For this review, take the finished solid that the model builds, in its own axes (mm). Face numbers are marked on the shaded views. A direction names the side the tool comes from. Coordinates: 2 decimals unless noted, no trailing zeros. Order: outer loops, then holes, each group sorted by start corner. A loop starts at its lowest first (then second) coordinate and runs counter-clockwise, first axis right, second up. Notation, with made-up numbers: (25, 18.25) -> (61, 18.25) arc R28 ccw to (61, 48.25) -> close; hole circle Ø1 at (-39.75, 7.25). An arc over 180 degrees is marked (long way). Answer as a JSON object with one key per item and string values. Group by question number.
1) Add section B-B, the plane x = 0. Write out the cut boundary in (y, z), then the cut area to 3 significant figures.
2) Draft analysis for pull direction X (two halves, no side actions). For the marked faces 1, 2 and 3, state which applies: +X half, -X half, draft (parallel to the pull), parting line (faces both ways), or undercut.
3) For pin 1 (4 mm diameter, centred on x = 20.5, y = 9, fed in from -Z); pin 2 (4 mm diameter, centred on x = 13.5, y = 18, fed in from -Z); pin 3 (5 mm diameter, centred on y = 4.5, z = 19, fed in from +X); pin 4 (15 mm diameter, centred on x = 0, z = 0, fed in from +Y), all flat-tipped, find the tip position at first contact; note any pin that passes through.
4) Machinability: for the marked faces 4 and 5, which of the approach directions +Z, -Z, +X, -X, +Y, -Y give a long, thin tool a straight path to every point of the face, cutting with its end or side? Answer none if there is none.
5) Add section D-D, the plane y = 17. Write out the cut boundary in (x, z).
6) Add section C-C, the plane y = 5.25. Write out the cut boundary in (x, z).
7) Add section A-A, the plane z = 0. Write out the cut boundary in (x, y).
8) Wall thickness on L1, parallel to Y at x = 12.5, z = 12; L2, parallel to Y at x = -13, z = -25.5; L3, parallel to X at y = 12.5, z = 0: over which ranges is each line inside the solid? List them lowest first.
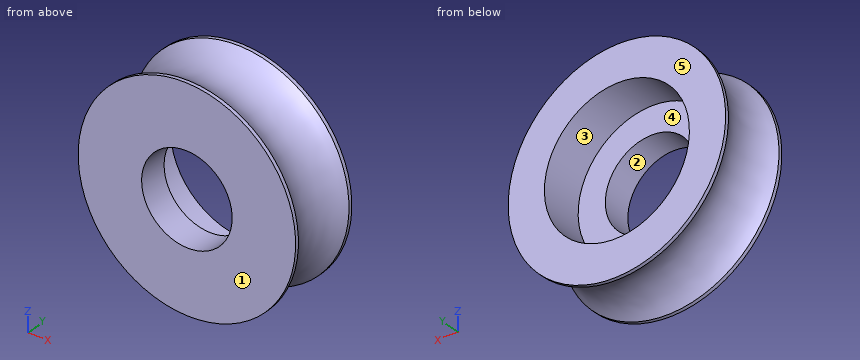
from build123d import *

# Parameters (mm, degrees)
SKETCH_1_R               = 30
EXTRUDE_1_DEPTH          = 20
SKETCH_2_R               = 20
CUT_EXTRUDE_1_DEPTH      = 12
CUT_EXTRUDE_2_DEPTH      = 45.09081537
CUT_EXTRUDE_2_DEPTH_BACK = 45.09081537
SKETCH_4_R               = 12.5
SKETCH_5_R               = 15


with BuildPart() as part:
    # 草图1 → 凸台-拉伸1 (new body)
    with BuildSketch(Plane(origin=(0, 0, 0), x_dir=(1, 0, 0), z_dir=(0, 1, 0))):
        with Locations(Location((0, 0, 0), (0, 0, 270))):
            Circle(SKETCH_1_R)
    extrude(amount=EXTRUDE_1_DEPTH)

    # 草图2 → 切除-拉伸1 (cut)
    with BuildSketch(Plane(origin=(0, 20, 0), x_dir=(1, 0, 0), z_dir=(0, 1, 0))):
        with Locations(Location((0, 0, 0), (0, 0, 270))):
            Circle(SKETCH_2_R)
    extrude(amount=-CUT_EXTRUDE_1_DEPTH, mode=Mode.SUBTRACT)

    # 草图4 → 切除-拉伸2 (cut, two sides: drawn at the far end of the back side and taken through both)
    with BuildSketch(Plane(origin=(0, 8, 0), x_dir=(1, 0, 0), z_dir=(0, 1, 0)).offset(-CUT_EXTRUDE_2_DEPTH_BACK)):
        with Locations(Location((0, 0, 0), (0, 0, 270))):
            Circle(SKETCH_4_R)
    extrude(amount=CUT_EXTRUDE_2_DEPTH + CUT_EXTRUDE_2_DEPTH_BACK, mode=Mode.SUBTRACT)

    # 草图5 → 切除-旋转1 (revolve, cut)
    with BuildSketch(Plane.XY, mode=Mode.PRIVATE) as cut_revolve_1_sk:
        with Locations((42, 10)):
            Circle(SKETCH_5_R)
    revolve(cut_revolve_1_sk.sketch.rotate(Axis((0, 0, 0), (0, 1, 0)), 90), axis=Axis((0, 0, 0), (0, 1, 0)), mode=Mode.SUBTRACT)


solid = part.part
Output values:
{
 "1": {"outline": "(0, -30) -> (1, -30) arc R15 cw to (19, -30) -> (20, -30) -> (20, -20) -> (8, -20) -> (8, -12.5) -> (0, -12.5) -> close; (0, 12.5) -> (8, 12.5) -> (8, 20) -> (20, 20) -> (20, 30) -> (19, 30) arc R15 cw to (1, 30) -> (0, 30) -> close", "area": "446 mm²"},
 "2": {"face 1": "draft", "face 2": "undercut", "face 3": "undercut"},
 "3": {"pin 1": "stops at z = -19.72", "pin 2": "stops at z = -27.6", "pin 3": "stops at x = 23.18", "pin 4": "passes through"},
 "4": {"face 4": "+Y", "face 5": "+Z, -Z, +X, -X, +Y"},
 "5": {"outline": "circle Ø57.47 at (0, 0); hole circle Ø40 at (0, 0)"},
 "6": {"outline": "circle Ø55.54 at (0, 0); hole circle Ø25 at (0, 0)"},
 "7": {"outline": "(-30, 0) -> (-12.5, 0) -> (-12.5, 8) -> (-20, 8) -> (-20, 20) -> (-30, 20) -> (-30, 19) arc R15 cw to (-30, 1) -> close; (12.5, 0) -> (30, 0) -> (30, 1) arc R15 cw to (30, 19) -> (30, 20) -> (20, 20) -> (20, 8) -> (12.5, 8) -> close"},
 "8": {"L1": "y = 0 to 8", "L2": "y = 0 to 3.21, 16.79 to 20", "L3": "x = -27.21 to -20, 20 to 27.21"}
}
